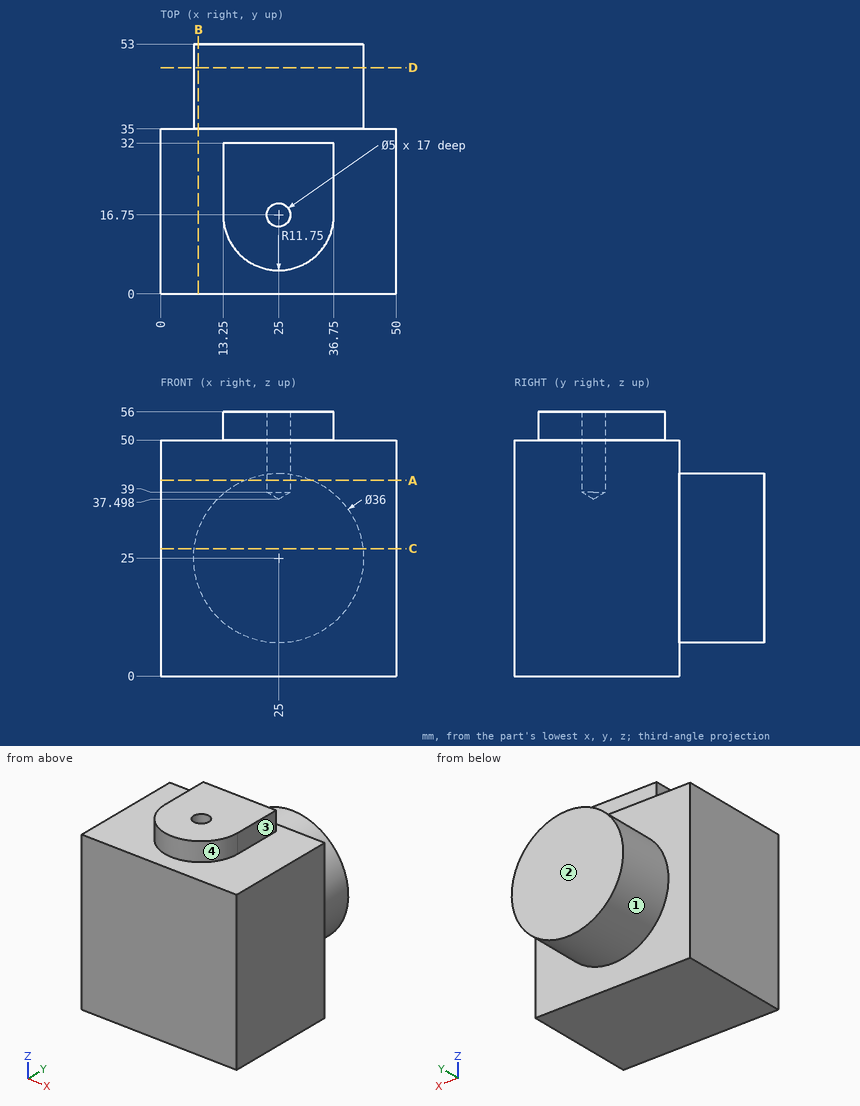
Check sheet for the drawn part. Datum: minimum x, y, z corner. Units: mm. A direction names the side the tool comes from. Coordinates: 2 decimals unless noted, no trailing zeros. Write each loop counter-clockwise with the first axis right and the second up, starting at its lowest first coordinate (ties: lowest second). Pieces come first, ordered by that corner, then holes. Notation, with made-up numbers: (84.25, 69.25) - (103.25, 69.25) arc R5 cw to (103.25, 75.25) - close; hole circle Ø8 at (49.25, 6). An arc over 180 degrees is marked (long way). Answer as a JSON object with one key per item and string values.
(1) Cross-section at C-C on z = 27. Record the cut outline in (x, y), plus the area to 3 significant figures.
Report:
{"outline": "(0, 0) - (50, 0) - (50, 35) - (42.89, 35) - (42.89, 53) - (7.11, 53) - (7.11, 35) - (0, 35) - close", "area": "2,390 mm^2"}
(2) Tool access check on the marked faces 1, 2, 3 and 4. Record the directions out of +Z, -Z, +X, -X, +Y, -Y that give a thin tool (end or side, any length) a straight path to the whole face; none if there is none.
Report:
{"face 1": "+Y", "face 2": "+Z, -Z, +X, -X, +Y", "face 3": "+Z, +X, +Y, -Y", "face 4": "+Z, -Y"}
(3) Thickness scan on line 1 along Y through (x, z) = (25, 46.75); line 2 along X through (y, z) = (16.75, 47); line 3 along Z through (x, y) = (37, 34.5). Record the ranges inside material, lowest first.
Report:
{"line 1": "0 to 14.25, 19.25 to 35", "line 2": "0 to 22.5, 27.5 to 50", "line 3": "0 to 50"}
(4) Gauge pin test, flat ends, axial feed: pin 1 Ø1.8 at (y, z) = (21.5, 52.5) entering from -X; pin 2 Ø6 at (y, z) = (10.5, 14.5) entering from -X; pin 3 Ø1.8 at (x, z) = (25.5, 53.5) entering from +Y; pin 4 Ø3 at (y, z) = (26.5, 54) entering from +X. Record the tip position at first contact, or that the pin passes through.
Report:
{"pin 1": "x = 13.25", "pin 2": "x = 0", "pin 3": "y = 32", "pin 4": "x = 36.75"}
(5) Cross-section at A-A on z = 41.5. Record the cut outline in (x, y), plus the area to 3 significant figures.
Report:
{"outline": "(0, 0) - (50, 0) - (50, 35) - (32.19, 35) - (32.19, 53) - (17.81, 53) - (17.81, 35) - (0, 35) - close; hole circle Ø5 at (25, 16.75)", "area": "1,990 mm^2"}
(6) Cross-section at D-D on y = 48. Record the cut outline in (x, z).
Report:
{"outline": "circle Ø36 at (25, 25)"}
(7) Cross-section at B-B on x = 8. Record the cut outline in (y, z).
Report:
{"outline": "(0, 0) - (35, 0) - (35, 19.08) - (53, 19.08) - (53, 30.92) - (35, 30.92) - (35, 50) - (0, 50) - close"}
